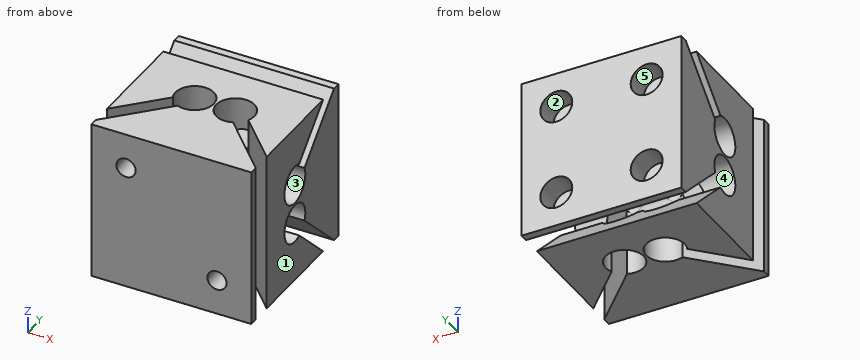
```python
from build123d import *

# Parameters (mm, degrees)
SKETCH1_W           = 10
SKETCH1_H           = 10
BOSS_EXTRUDE1_DEPTH = 10
CUT_EXTRUDE1_DEPTH  = 16
CUT_EXTRUDE2_DEPTH  = 16
SKETCH5_R           = 0.6
CUT_EXTRUDE3_DEPTH  = 2
SKETCH6_R           = 1
CUT_EXTRUDE4_DEPTH  = 1.5


with BuildPart() as part:
    # Sketch1 → Boss-Extrude1 (new body)
    with BuildSketch(Plane(origin=(0, 0, 0), x_dir=(1, 0, 0), z_dir=(0, 1, 0))):
        Rectangle(SKETCH1_W, SKETCH1_H)
    extrude(amount=BOSS_EXTRUDE1_DEPTH)

    # Sketch2 → Cut-Extrude1 (cut, through all)
    with BuildSketch(Plane.XY.offset(5)):
        with BuildLine():
            Line((2.363818154, 4.495544821), (5, 1.754964793))
            Line((5, 1.754964793), (5, 0.5))
            Line((5, 0.5), (1.736808704, 3.892420332))
            ThreePointArc((1.736808704, 3.892420332), (0.443104153, 5.864840621), (2.363818154, 4.495544821))
        make_face()
        with BuildLine():
            Line((-5, 1.754964793), (-5, 0.5))
            Line((-5, 0.5), (-1.736808704, 3.892420332))
            ThreePointArc((-1.736808704, 3.892420332), (-0.443104153, 5.864840621), (-2.363818154, 4.495544821))
            Line((-2.363818154, 4.495544821), (-5, 1.754964793))
        make_face()
    extrude(amount=-CUT_EXTRUDE1_DEPTH, mode=Mode.SUBTRACT)

    # Sketch3 → Cut-Extrude2 (cut, through all)
    with BuildSketch(Plane(origin=(5, 0, 0), x_dir=(0, 0, -1), z_dir=(1, 0, 0))):
        with BuildLine():
            Line((2.363818154, 5.504455179), (5, 8.245035207))
            Line((5, 8.245035207), (5, 9.5))
            Line((5, 9.5), (1.736808704, 6.107579668))
            ThreePointArc((1.736808704, 6.107579668), (0.443104153, 4.135159379), (2.363818154, 5.504455179))
        make_face()
        with BuildLine():
            Line((-5, 9.5), (-5, 8.245035207))
            Line((-5, 8.245035207), (-2.363818154, 5.504455179))
            ThreePointArc((-2.363818154, 5.504455179), (-0.443104153, 4.135159379), (-1.736808704, 6.107579668))
            Line((-1.736808704, 6.107579668), (-5, 9.5))
        make_face()
    extrude(amount=-CUT_EXTRUDE2_DEPTH, mode=Mode.SUBTRACT)

    # Sketch5 → Cut-Extrude3 (cut)
    with BuildSketch(Plane.XZ):
        with Locations(Location((-2.84590029, 2.810845343, 0), (0, 0, 270))):
            Circle(SKETCH5_R)
        with Locations(Location((2.84590029, -2.810845343, 0), (0, 0, 270))):
            Circle(SKETCH5_R)
    extrude(amount=-CUT_EXTRUDE3_DEPTH, mode=Mode.SUBTRACT)

    # Sketch6 → Cut-Extrude4 (cut)
    with BuildSketch(Plane(origin=(0, 10, 0), x_dir=(1, 0, 0), z_dir=(0, 1, 0))):
        with Locations(Location((-2.828427125, 2.828427125, 0), (0, 0, 270))):
            Circle(SKETCH6_R)
        with Locations(Location((2.828427125, 2.828427125, 0), (0, 0, 270))):
            Circle(SKETCH6_R)
        with Locations(Location((2.828427125, -2.828427125, 0), (0, 0, 270))):
            Circle(SKETCH6_R)
        with Locations(Location((-2.828427125, -2.828427125, 0), (0, 0, 270))):
            Circle(SKETCH6_R)
    extrude(amount=-CUT_EXTRUDE4_DEPTH, mode=Mode.SUBTRACT)


solid = part.part
```
CAD build for the part. Positions are in the model's coordinates, mm. Face numbers are marked on the shaded views. A direction names the side the tool comes from. Coordinates: 2 decimals unless noted, no trailing zeros. Order: outer loops, then holes, each group sorted by start corner. A loop starts at its lowest first (then second) coordinate and runs counter-clockwise, first axis right, second up. Notation, with made-up numbers: (12, 19.5) - (28, 19.5) arc R14 cw to (28, 25.5) - close; hole circle Ø3 at (-26, -20.75). An arc over 180 degrees is marked (long way). Use a Markdown table: item, result. Add a question column.
(1) Drill centre lines: line 1 along Z through (x, y) = (3.1, 5) (3 decimals); line 2 along Y through (x, z) = (-0.5, 1.25); line 3 along Y through (x, z) = (-4.25, 2.25). Where is each one in solid material? Low to high. Write a range as [from, to].
(2) Pull direction X, two halves, no side cores. Call the marked faces 1, 2 and 3: +X half, -X half, draft (parallel to the pull), parting line (faces both ways), or undercut.
(3) Which spindle directions (+Z, -Z, +X, -X, +Y, -Y) get a long thin tool onto all of the face, cutting with end or side? Do the marked faces 4 and 5. Say none if no direction does.
(4) Saw through at C-C (x = 4). Give the cut face in (y, z) (3 decimals), then the cut area to 3 significant figures.
(5) Saw through at A-A (y = 3.25). Give the cut face in (x, z).
(6) Flat gauge pins, fed straight in: pin 1 (2 mm diameter, centred on y = 5, z = -1.275, fed in from -X); pin 2 (1 mm diameter, centred on x = 3, z = 2.5, fed in from +Y). Where does each tip first touch, or does it go through?
(7) Saw through at D-D (x = 1.5). Give the cut face in (y, z) (3 decimals).
(8) Saw through at B-B (z = -0.5). Give the cut face in (x, y) (3 decimals).
Solved:
| question | item | result |
|---|---|---|
| 1 | line 1 | z = [-5, -2.475], [-0.075, 0.075], [2.475, 5] |
| 1 | line 2 | y = [0, 3.8], [6.2, 10] |
| 1 | line 3 | y = [0, 1.28], [2.53, 4.3], [6.64, 10] |
| 2 | face 1 | +X half |
| 2 | face 2 | undercut |
| 2 | face 3 | draft |
| 3 | face 4 | +X, -X |
| 3 | face 5 | +Y |
| 4 | outline | (0, -5) - (1.54, -5) - (1.54, 5) - (0, 5) - close; (2.795, -5) - (8.245, -5) - (5.504, -2.364) arc R1.2 cw (long way) to (6.108, -1.737) - (9.5, -5) - (10, -5) - (10, 5) - (9.5, 5) - (6.108, 1.737) arc R1.2 cw (long way) to (5.504, 2.364) - (8.245, 5) - (2.795, 5) - close |
| 4 | area | 71.1 mm² |
| 5 | outline | (-5, -5) - (-3.56, -5) - (-3.56, 5) - (-5, 5) - close; (-2.35, -5) - (2.35, -5) - (2.35, 5) - (-2.35, 5) - close; (3.56, -5) - (5, -5) - (5, 5) - (3.56, 5) - close |
| 6 | pin 1 | passes through |
| 6 | pin 2 | stops at y = 8.5 |
| 7 | outline | (0, -5) - (3.821, -5) - (3.821, -1.5) arc R1.2 cw to (3.821, -1.05) - (3.821, 1.05) arc R1.2 cw to (3.821, 1.5) - (3.821, 5) - (0, 5) - close; (6.179, -5) - (8.245, -5) - (6.179, -3.012) - close; (6.179, -1.805) - (9.5, -5) - (10, -5) - (10, 5) - (9.5, 5) - (6.179, 1.805) - (6.179, 1.5) arc R1.2 cw to (6.179, 1.05) - (6.179, -1.05) arc R1.2 cw to (6.179, -1.5) - close; (6.179, 3.012) - (8.245, 5) - (6.179, 5) - close |
| 8 | outline | (-5, 0) - (5, 0) - (5, 0.5) - (1.737, 3.892) arc R1.2 cw to (0.5, 4.084) - (-0.5, 4.084) arc R1.2 cw to (-1.737, 3.892) - (-5, 0.5) - close; (-5, 1.755) - (-2.76, 4.084) - (-5, 4.084) - close; (-5, 5.916) - (-2.05, 5.916) arc R1.2 cw to (-0.5, 5.916) - (0.5, 5.916) arc R1.2 cw to (2.05, 5.916) - (5, 5.916) - (5, 10) - (-5, 10) - close; (2.76, 4.084) - (5, 1.755) - (5, 4.084) - close |
